Study the drawing (mm; zero at the part's minimum x, y, z) and answer. A direction names the side the tool comes from. Round coordinates to 2 decimals unless told otherwise and drop trailing zeros. Loops run counter-clockwise (first coordinate to the right, second up) from the corner with the lowest first, then second, coordinate; pieces in that order, holes last. Notation, with made-up numbers: (70.5, 45) -> (122.5, 45) arc R22 ccw to (122.5, 62) -> close; hole circle Ø2 at (67.5, 24.5). An arc over 180 degrees is marked (long way). Write each question's results on one line, items separated by ' | '. Start each with the question number.
(1) A flat-ended cylindrical pin translates along its axis: pin 1 (3.5 mm diameter, centred on x = 10, y = 13, fed in from +Z). Find the tip coordinate at first contact, or state that the pin passes through.
(2) The part is cut by section D-D (z = 2.5). Determine the outline of the cut face in (x, y), plus the area to 3 significant figures.
(3) Determine the mould class of the marked faces 1, 2 and 3 for opening direction X: released by +X, released by -X, zero draft, split by the parting line, or undercut.
(4) The part is cut by section A-A (y = 2.5). Determine the outline of the cut face in (x, z).
(5) Straight lines are drawn through the part: probe 1 along Y at (x, z) = (3, 1.45); probe 2 along Y at (x, z) = (16.25, 2.1); probe 3 along Y at (x, z) = (10, 1.9). For each, find the intervals that lie inside material, in ascending order.
(6) The part is cut by section B-B (x = 10). Determine the outline of the cut face in (y, z), plus the area to 3 significant figures.
(7) For the marked faces 4 and 5, determine the directions among +Z, -Z, +X, -X, +Y, -Y from which every point of the face is accessible in a straight line to the end or side of a thin tool.
(8) The part is cut by section C-C (y = 20). Determine the outline of the cut face in (x, z), plus the area to 3 significant figures.
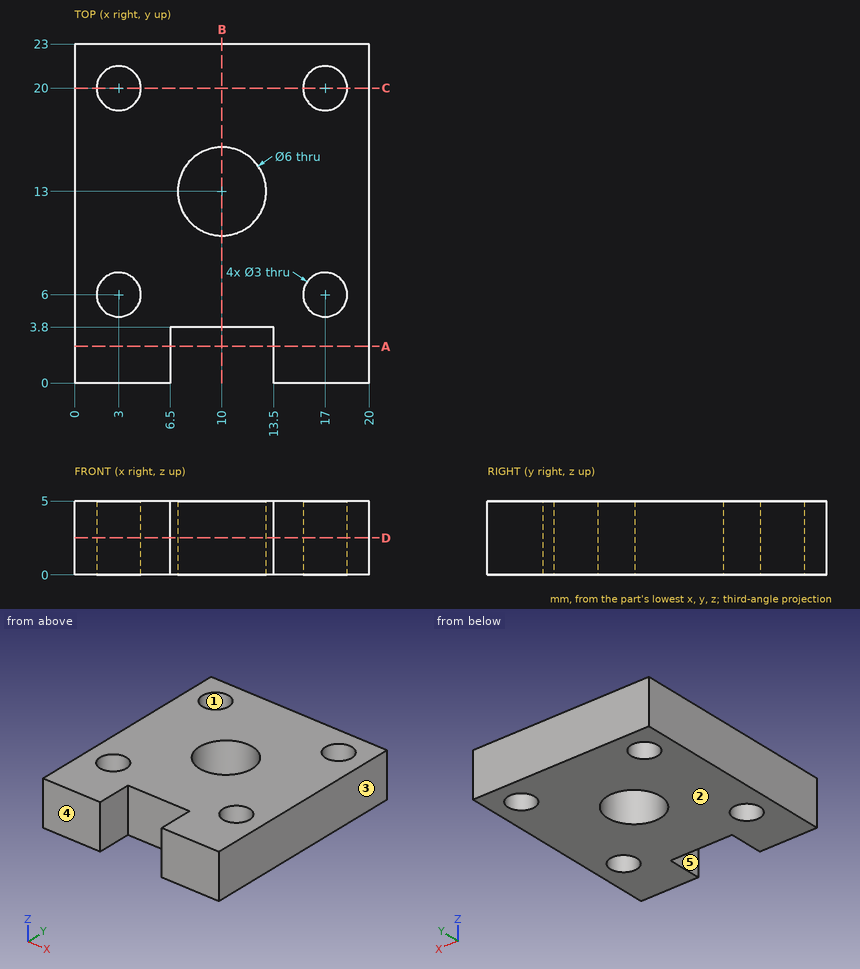
Checked values:
1) pin 1: passes through
2) outline: (0, 0) -> (6.5, 0) -> (6.5, 3.8) -> (13.5, 3.8) -> (13.5, 0) -> (20, 0) -> (20, 23) -> (0, 23) -> close; hole circle Ø3 at (3, 6); hole circle Ø3 at (3, 20); hole circle Ø6 at (10, 13); hole circle Ø3 at (17, 6); hole circle Ø3 at (17, 20) | area: 377 mm2
3) face 1: undercut | face 2: zero draft | face 3: released by +X
4) outline: (0, 0) -> (6.5, 0) -> (6.5, 5) -> (0, 5) -> close; (13.5, 0) -> (20, 0) -> (20, 5) -> (13.5, 5) -> close
5) probe 1: y = 0 to 4.5, 7.5 to 18.5, 21.5 to 23 | probe 2: y = 0 to 4.7, 7.3 to 18.7, 21.3 to 23 | probe 3: y = 3.8 to 10, 16 to 23
6) outline: (3.8, 0) -> (10, 0) -> (10, 5) -> (3.8, 5) -> close; (16, 0) -> (23, 0) -> (23, 5) -> (16, 5) -> close | area: 66.0 mm2
7) face 4: +Z, -Z, +X, -X, -Y | face 5: +Z, -Z, -Y
8) outline: (0, 0) -> (1.5, 0) -> (1.5, 5) -> (0, 5) -> close; (4.5, 0) -> (15.5, 0) -> (15.5, 5) -> (4.5, 5) -> close; (18.5, 0) -> (20, 0) -> (20, 5) -> (18.5, 5) -> close | area: 70.0 mm2
